The listing builds one solid part. Answer for the finished solid, in the listing's coordinates (mm). A direction names the side the tool comes from. Round coordinates to 2 decimals unless told otherwise and drop trailing zeros. Order: outer loops, then holes, each group sorted by start corner. A loop starts at its lowest first (then second) coordinate and runs counter-clockwise, first axis right, second up. Notation, with made-up numbers: (-17.75, 85.5) -> (17.25, 85.5) arc R21 ccw to (17.25, 112.5) -> close; hole circle Ø8 at (74, 29.25). An arc over 180 degrees is marked (long way). Return JSON: item names as keys, results as strings. Group by question number.
(1) The part is cut by section D-D (x = 96.5). Determine the outline of the cut face in (y, z), plus the area to 3 significant figures.
(2) Consider line 1 (X direction, y = 16, z = 0); line 2 (X direction, y = 31, z = -2.5); line 3 (Z direction, x = 96, y = 6). Determine where each line is inside the solid, lowest interval first. Write a range as [from, to].
(3) Which of the six approach directions +Z, -Z, +X, -X, +Y, -Y give full straight-line access (tool end or side, diameter ignored) to faces 5 (the face through (136.16, 12.32, 5.21)), 6 (the face through (-2, 40, -27))?
(4) The part is cut by section A-A (z = 0). Determine the outline of the cut face in (x, y), plus the area to 3 significant figures.
(5) The part is cut by section C-C (y = 7). Determine the outline of the cut face in (x, z).
(6) Determine the mould class of faces 1 (the face through (-45.287, 19.72, 6.503)), 2 (the face through (131.2, 32.39, 4.56)), 3 (the face through (-2, 20, -112.5)), 4 (the face through (-2, 0, -27)) for opening direction Z: +Z half, -Z half, draft (parallel to the pull), parting line (faces both ways), or undercut.
(7) The part is cut by section B-B (x = -16). Determine the outline of the cut face in (y, z).
from build123d import *

# Parameters (mm, degrees)
SKETCH_1_W          = 293
SKETCH_1_H          = 225
EXTRUDE_1_DEPTH     = 40
SKETCH_2_R          = 40
CUT_EXTRUDE_1_DEPTH = 25
SKETCH_3_R          = 30
CUT_EXTRUDE_2_DEPTH = 189.993386128
SKETCH_4_R          = 35
CUT_EXTRUDE_3_DEPTH = 189.993386128


with BuildPart() as part:
    # 草图1 → 凸台-拉伸1 (new body)
    with BuildSketch(Plane(origin=(0, 0, 0), x_dir=(1, 0, 0), z_dir=(0, 1, 0))):
        Rectangle(SKETCH_1_W, SKETCH_1_H)
    extrude(amount=EXTRUDE_1_DEPTH)

    # 草图2 → 切除-拉伸1 (cut)
    with BuildSketch(Plane.XZ):
        with Locations(Location((96.5, 0, 0), (0, 0, 270))):
            Circle(SKETCH_2_R)
    extrude(amount=-CUT_EXTRUDE_1_DEPTH, mode=Mode.SUBTRACT)

    # 草图3 → 切除-拉伸2 (cut, through all)
    with BuildSketch(Plane.XZ):
        with Locations(Location((-16, 0, 0), (0, 0, 270))):
            Circle(SKETCH_3_R)
    extrude(amount=-CUT_EXTRUDE_2_DEPTH, mode=Mode.SUBTRACT)

    # 草图4 → 切除-拉伸3 (cut, through all)
    with BuildSketch(Plane.XZ):
        with Locations(Location((96.5, 0, 0), (0, 0, 270))):
            Circle(SKETCH_4_R)
    extrude(amount=-CUT_EXTRUDE_3_DEPTH, mode=Mode.SUBTRACT)


solid = part.part
Answer below:
{
 "1": {"outline": "(0, -112.5) -> (40, -112.5) -> (40, -35) -> (25, -35) -> (25, -40) -> (0, -40) -> close; (0, 40) -> (25, 40) -> (25, 35) -> (40, 35) -> (40, 112.5) -> (0, 112.5) -> close", "area": "5,950 mm²"},
 "2": {"line 1": "x = [-146.5, -46], [14, 56.5], [136.5, 146.5]", "line 2": "x = [-146.5, -45.9], [13.9, 61.59], [131.41, 146.5]", "line 3": "z = [-112.5, -40], [40, 112.5]"},
 "3": {"face 5": "-Y", "face 6": "+Z, -Z, +X, -X, +Y"},
 "4": {"outline": "(-146.5, 0) -> (-46, 0) -> (-46, 40) -> (-146.5, 40) -> close; (14, 0) -> (56.5, 0) -> (56.5, 25) -> (61.5, 25) -> (61.5, 40) -> (14, 40) -> close; (131.5, 25) -> (136.5, 25) -> (136.5, 0) -> (146.5, 0) -> (146.5, 40) -> (131.5, 40) -> close", "area": "6,270 mm²"},
 "5": {"outline": "(-146.5, -112.5) -> (146.5, -112.5) -> (146.5, 112.5) -> (-146.5, 112.5) -> close; hole circle Ø60 at (-16, 0); hole circle Ø80 at (96.5, 0)"},
 "6": {"face 1": "undercut", "face 2": "undercut", "face 3": "-Z half", "face 4": "draft"},
 "7": {"outline": "(0, -112.5) -> (40, -112.5) -> (40, -30) -> (0, -30) -> close; (0, 30) -> (40, 30) -> (40, 112.5) -> (0, 112.5) -> close"}
}
